```python
from build123d import *

# Parameters (mm, degrees)
SKETCH1_W            = 35
SKETCH1_H            = 5
BOSS_EXTRUDE3_DEPTH  = 5
SKETCH7_W            = 5
SKETCH7_H            = 5
BOSS_EXTRUDE6_DEPTH  = 5
FILLET6_R            = 1
FILLET7_R            = 1
SKETCH11_R           = 2
CUT_EXTRUDE2_DEPTH   = 5
SKETCH5_R            = 2.375
BOSS_EXTRUDE9_DEPTH  = 5
SKETCH13_R           = 4
BOSS_EXTRUDE10_DEPTH = 5
SKETCH14_R           = 2.625
CUT_EXTRUDE3_DEPTH   = 25.84321589
SKETCH15_W           = 5
SKETCH15_H           = 5
BOSS_EXTRUDE11_DEPTH = 0.875
FILLET8_R            = 2
FILLET9_R            = 2
SKETCH16_R           = 4
BOSS_EXTRUDE12_DEPTH = 5
SKETCH17_R           = 2.625
CUT_EXTRUDE4_DEPTH   = 30
CUT_EXTRUDE5_DEPTH   = 25.84321589
BOSS_EXTRUDE13_DEPTH = 5


with BuildPart() as part:
    # Sketch1 → Boss-Extrude3 (new body)
    with BuildSketch(Plane.XY):
        Rectangle(SKETCH1_W, SKETCH1_H)
    extrude(amount=BOSS_EXTRUDE3_DEPTH)

    # Sketch7 → Boss-Extrude6 (add)
    with BuildSketch(Plane.XY.offset(5)):
        with Locations((20, 0.046210476)):
            Rectangle(SKETCH7_W, SKETCH7_H)
    extrude(amount=-BOSS_EXTRUDE6_DEPTH)

    # Fillet6
    fillet6_edges = [part.edges().sort_by_distance(p)[0] for p in [
        (22.5, 2.546210476, 2.5),
    ]]
    fillet(fillet6_edges, radius=FILLET6_R)

    # Fillet7
    fillet7_edges = [part.edges().sort_by_distance(p)[0] for p in [
        (22.5, -2.453789524, 2.5),
    ]]
    fillet(fillet7_edges, radius=FILLET7_R)

    # Sketch11 → Cut-Extrude2 (cut)
    with BuildSketch(Plane.XY.offset(5)):
        with Locations((20, 0.023105238)):
            Circle(SKETCH11_R)
    extrude(amount=-CUT_EXTRUDE2_DEPTH, mode=Mode.SUBTRACT)

    # Sketch5 → Boss-Extrude9 (add)
    with BuildSketch(Plane.XY.offset(5)):
        with Locations(Location((-16, 0, 0), (0, 0, 230.833289284))):
            Circle(SKETCH5_R)
    extrude(amount=BOSS_EXTRUDE9_DEPTH)

    # Sketch13 → Boss-Extrude10 (add, through all)
    with BuildSketch(Plane.XY.offset(5)):
        with Locations((20, 0.023105238)):
            Circle(SKETCH13_R)
    extrude(amount=-BOSS_EXTRUDE10_DEPTH)

    # Sketch14 → Cut-Extrude3 (cut, through all)
    with BuildSketch(Plane.XY.offset(5)):
        with Locations((20, 0.023105238)):
            Circle(SKETCH14_R)
    extrude(amount=-CUT_EXTRUDE3_DEPTH, mode=Mode.SUBTRACT)

    # Sketch15 → Boss-Extrude11 (add, through all)
    with BuildSketch(Plane.ZY.offset(17.5)):
        with Locations((2.5, 0)):
            Rectangle(SKETCH15_W, SKETCH15_H)
    extrude(amount=BOSS_EXTRUDE11_DEPTH)

    # Fillet8
    fillet8_edges = [part.edges().sort_by_distance(p)[0] for p in [
        (-18.375, 2.5, 2.5),
    ]]
    fillet(fillet8_edges, radius=FILLET8_R)

    # Fillet9
    fillet9_edges = [part.edges().sort_by_distance(p)[0] for p in [
        (-18.375, -2.5, 2.5),
    ]]
    fillet(fillet9_edges, radius=FILLET9_R)

    # Sketch16 → Boss-Extrude12 (add)
    with BuildSketch(Plane.XY.offset(5)):
        with Locations((-16, 0)):
            Circle(SKETCH16_R)
    extrude(amount=-BOSS_EXTRUDE12_DEPTH)

    # Sketch17 → Cut-Extrude4 (cut)
    with BuildSketch(Plane.XY.offset(10)):
        with Locations(Location((-16, 0, 0), (0, 0, 180))):
            Circle(SKETCH17_R)
    extrude(amount=-CUT_EXTRUDE4_DEPTH, mode=Mode.SUBTRACT)

    # Sketch18 → Cut-Extrude5 (cut, through all)
    with BuildSketch(Plane.XY.offset(5)):
        with BuildLine():
            Line((-12, 0), (16, 0.023105238))
            ThreePointArc((16, 0.023105238), (17.170665329, 2.850624525), (19.99743266, 4.023104414))
            Line((19.99743266, 4.023104414), (-16, 4))
            ThreePointArc((-16, 4), (-13.171572875, 2.828427125), (-12, 0))
        make_face()
    extrude(amount=-CUT_EXTRUDE5_DEPTH, mode=Mode.SUBTRACT)

    # Sketch19 → Boss-Extrude13 (add, through all)
    with BuildSketch(Plane.XY.offset(5)):
        Polygon((-16, -4), (20, -3.976894762), (16, -1.273335264), (-12.878635235, -1.649219819), align=None)
    extrude(amount=-BOSS_EXTRUDE13_DEPTH)


solid = part.part
```
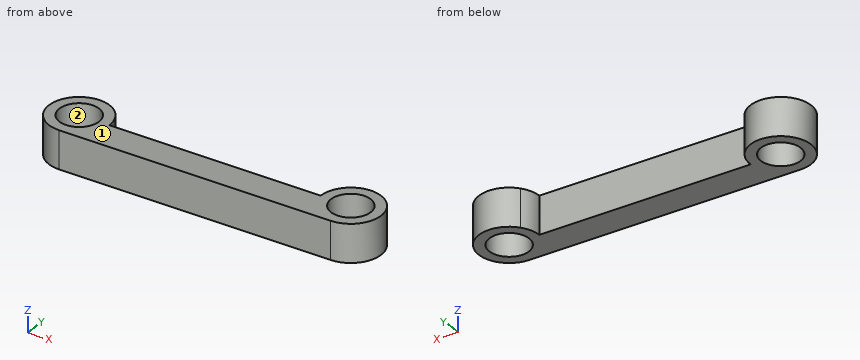
Can you work these out from the model? Positions are in its coordinate system, mm. Face numbers are marked on the shaded views. Give positions to 0.01 mm unless a question says otherwise; leave off trailing zeros. Write each loop counter-clockwise with the first axis right and the second up, starting at its lowest first coordinate (ties: lowest second). Pieces come first, ordered by that corner, then holes. Notation, with made-up numbers: (30.5, -19.75) -> (57.5, -19.75) arc R18 ccw to (57.5, 5.25) -> close; hole circle Ø3 at (-32, 34.25). An arc over 180 degrees is marked (long way). One line per item, written item: value.
Q1. We'd pull the mould along Y, two halves only. Please class the marked faces 1 and 2: +Y half, -Y half, draft (parallel to the pull), parting line (faces both ways), or undercut.
Results found:
face 1: draft
face 2: undercut
Q2. Please list where these lines run through material, in increasing order: line 1 (X direction, y = -1, z = 0.75); line 2 (X direction, y = -1.25, z = 1.25); line 3 (X direction, y = 1.5, z = 2.8). Write a range as [from, to].
Results found:
line 1: x = [-19.87, -18.43], [-13.57, 17.58], [22.42, 23.87]
line 2: x = [-19.8, -18.31], [-13.69, 17.7], [22.3, 23.79]
line 3: x = [-19.71, -18.15], [-13.85, -12.29], [16.28, 17.83], [22.17, 23.72]
Q3. Imagine slicing it at D-D on x = -7. Please give me the cut outline in (y, z), and give its area (3 significant figures).
Results found:
outline: (-3.99, 0) -> (0, 0) -> (0, 5) -> (-3.99, 5) -> close
area: 20.0 mm^2
Q4. For P1, Ø3, axis at x = 6, z = 2.5, coming from the -Y side; P2, Ø4, axis at x = 11.5, y = 3, coming from the -Z side; P3, Ø1.5, axis at y = 2, z = 1.5, coming from the -X side, each with a flat end and sliding along its axis, tell me the tip position at first contact or that it passes through.
Results found:
P1: stops at y = -3.99
P2: passes through
P3: stops at x = -19.8
Q5. Imagine slicing it at B-B on y = 1.25. Please give me the cut outline in (x, z), and give its area (3 significant figures).
Results found:
outline: (-19.8, 0) -> (-18.31, 0) -> (-18.31, 5) -> (-19.8, 5) -> close; (-13.69, 0) -> (-12.2, 0) -> (-12.2, 5) -> (-13.69, 5) -> close; (16.19, 0) -> (17.68, 0) -> (17.68, 5) -> (16.19, 5) -> close; (22.32, 0) -> (23.81, 0) -> (23.81, 5) -> (22.32, 5) -> close
area: 29.8 mm^2
Q6. Imagine slicing it at C-C on y = -0.5. Please give me the cut outline in (x, z).
Results found:
outline: (-19.97, 0) -> (-18.58, 0) -> (-18.58, 5) -> (-19.97, 5) -> close; (-13.42, 0) -> (17.43, 0) -> (17.43, 5) -> (-13.42, 5) -> close; (22.57, 0) -> (23.97, 0) -> (23.97, 5) -> (22.57, 5) -> close
Q7. Imagine slicing it at A-A on z = 1.6. Give the number of separate pieces and of enclosed holes in the cut face, and give its area (3 significant figures).
Results found:
separate pieces: 1
enclosed holes: 2
area: 176 mm^2
